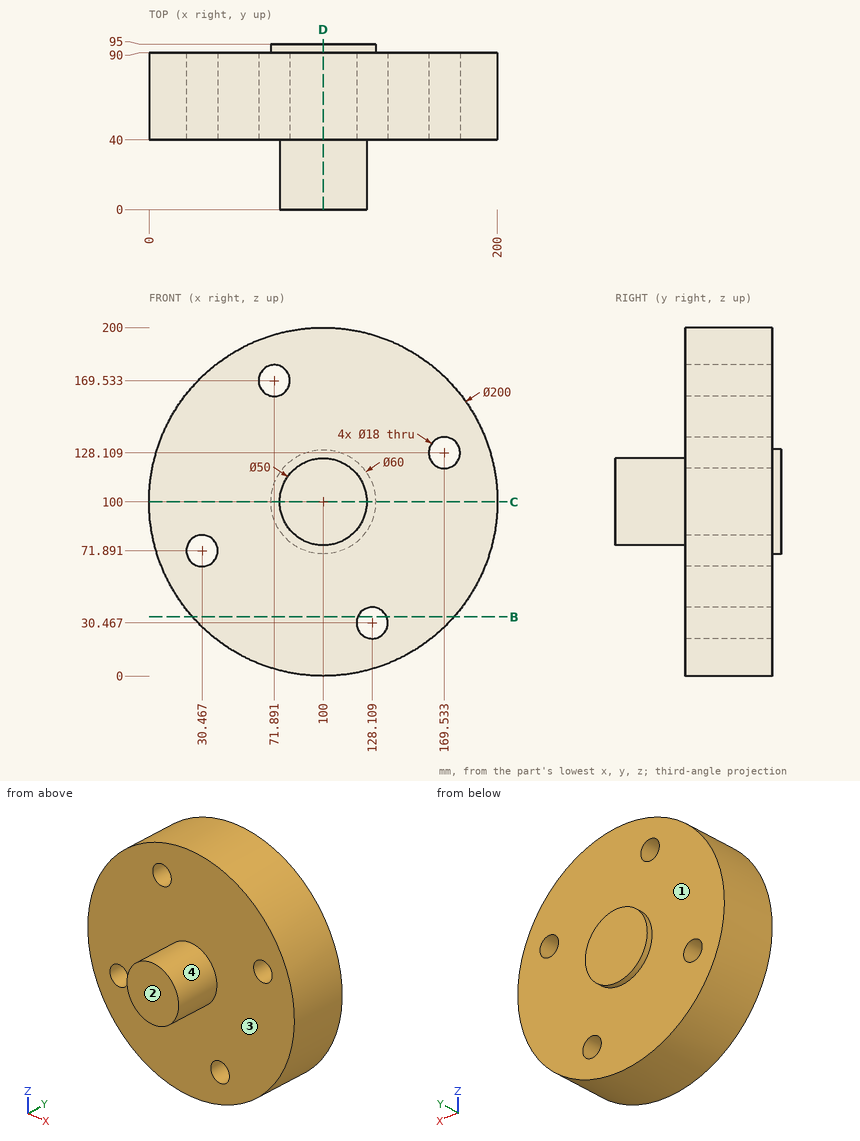
Study the drawing (mm; zero at the part's minimum x, y, z) and answer. A direction names the side the tool comes from. Coordinates: 2 decimals unless noted, no trailing zeros. Loops run counter-clockwise (first coordinate to the right, second up) from the corner with the lowest first, then second, coordinate; pieces in that order, holes last. Notation, with made-up numbers: (-7, 6.25) -> (51, 6.25) arc R25 ccw to (51, 25.25) -> close; hole circle Ø6 at (-37, 14.5). An arc over 180 degrees is marked (long way). Answer in a Markdown table with one row per item. Add a question column.
1. For the marked faces 1 and 2, determine the directions among +Z, -Z, +X, -X, +Y, -Y from which every point of the face is accessible in a straight line to the end or side of a thin tool.
2. The part is cut by section B-B, the plane z = 34. Write down the section's boundary in (x, y).
3. Consider line 1 (Y direction, x = 145, z = 95); line 2 (Z direction, x = 30, y = 75) (1 decimal); line 3 (X direction, y = 68, z = 120.5) (1 decimal). Determine where each line is inside the solid, lowest interval first. Write a range as [from, to].
4. Determine the mould class of the marked faces 3 and 4 for opening direction Z: +Z half, -Z half, draft (parallel to the pull), parting line (faces both ways), or undercut.
5. Flat-ended cylindrical pins translate along their axes: P1, Ø3, axis at y = 48.5, z = 66, coming from the +X side; P2, Ø14.5, axis at x = 128.11, z = 30.47, coming from the +Y side; P3, Ø3, axis at x = 158, y = 84, coming from the +Z side; P4, Ø6, axis at y = 71, z = 107, coming from the -X side. Find the tip coordinate at first contact, or state that the pin passes through.
6. The part is cut by section C-C, the plane z = 100. Write down the section's boundary in (x, y), then the cut area to 3 significant figures.
7. The part is cut by section D-D, the plane x = 100. Write down the section's boundary in (y, z).
Answer below:
| question | item | result |
|---|---|---|
| 1 | face 1 | +Y |
| 1 | face 2 | +Z, -Z, +X, -X, -Y |
| 2 | outline | (24.87, 40) -> (119.83, 40) -> (119.83, 90) -> (24.87, 90) -> close; (136.39, 40) -> (175.13, 40) -> (175.13, 90) -> (136.39, 90) -> close |
| 3 | line 1 | [40, 90] |
| 3 | line 2 | [28.6, 62.9], [80.9, 171.4] |
| 3 | line 3 | [2.1, 164.7], [174.3, 197.9] |
| 4 | face 3 | draft |
| 4 | face 4 | parting line |
| 5 | P1 | x = 194.57 |
| 5 | P2 | through |
| 5 | P3 | z = 182.51 |
| 5 | P4 | x = 0.08 |
| 6 | outline | (0, 40) -> (75, 40) -> (75, 0) -> (125, 0) -> (125, 40) -> (200, 40) -> (200, 90) -> (130, 90) -> (130, 95) -> (70, 95) -> (70, 90) -> (0, 90) -> close |
| 6 | area | 12,300 mm2 |
| 7 | outline | (0, 75) -> (40, 75) -> (40, 0) -> (90, 0) -> (90, 70) -> (95, 70) -> (95, 130) -> (90, 130) -> (90, 200) -> (40, 200) -> (40, 125) -> (0, 125) -> close |
